Source: CAD feature listing. Evaluate the final solid. Frame: model axes, mm. Face numbers are marked on the shaded views. A direction names the side the tool comes from. Coordinates: 2 decimals unless noted, no trailing zeros. Loops run counter-clockwise (first coordinate to the right, second up) from the corner with the lowest first, then second, coordinate; pieces in that order, holes last. Notation, with made-up numbers: M 78,7.5 L 129,7.5 A19 ccw 129,35.5 Z; hole C 54.25,-7.75 d10. An arc over 180 degrees is marked long. Write each question's results on one line, items separated by ' | '. Start each with the question number.
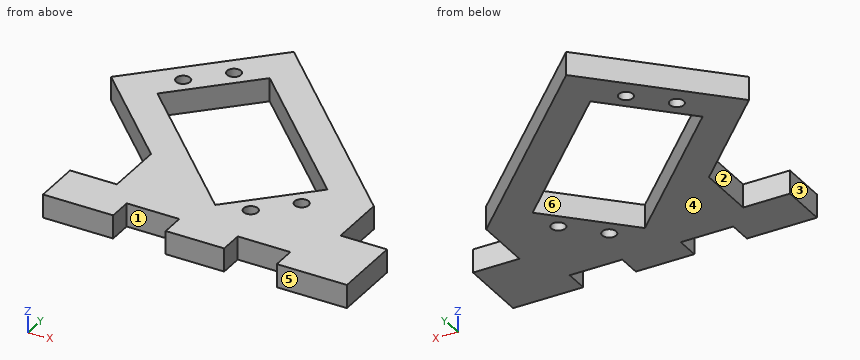
from build123d import *

# Parameters (mm, degrees)
SKETCH_1_R      = 1.5
EXTRUDE_1_DEPTH = 5


with BuildPart() as part:
    # 草图1 → 凸台-拉伸1 (new body)
    with BuildSketch(Plane.XY):
        Polygon((-12.648598414, -34.707783696), (-27.648598414, -34.707783696), (-27.648598414, -24.707783696), (-17.648598414, -24.707783696), (-17.648598414, -12.085840997), (-37.977918373, 8.243478962), (-13.229181032, 32.992216304), (27.420818968, -7.657783696), (27.420818968, -19.907783696), (37.351401586, -19.907783696), (37.351401586, -34.707783696), (22.351401586, -34.707783696), (22.351401586, -29.707783696), (11.101401586, -29.707783696), (11.101401586, -34.707783696), (-1.398598414, -34.707783696), (-1.398598414, -29.707783696), (-12.648598414, -29.707783696), align=None)
        with Locations((-19.009778968, 20.918368015)):
            Circle(SKETCH_1_R, mode=Mode.SUBTRACT)
        with Locations((-25.904070084, 14.024076898)):
            Circle(SKETCH_1_R, mode=Mode.SUBTRACT)
        with Locations((15.355610598, -13.447021551)):
            Circle(SKETCH_1_R, mode=Mode.SUBTRACT)
        with Locations((8.461319481, -20.341312667)):
            Circle(SKETCH_1_R, mode=Mode.SUBTRACT)
        Polygon((-27.548093351, 7.359595486), (1.796838069, -21.985335933), (16.999633864, -6.782540138), (-12.345297555, 22.562391281), align=None, mode=Mode.SUBTRACT)
    extrude(amount=EXTRUDE_1_DEPTH)


solid = part.part
Item 1: Line query: probe 1 along X at (y, z) = (-13.5, 3.6); probe 2 along Y at (x, z) = (-19.5, 0.85); probe 3 along X at (y, z) = (-28, 2). Output: solid intervals per line, ascending.
Item 2: Access query for the marked faces 1, 2 and 3. Directions: +Z, -Z, +X, -X, +Y, -Y. A direction counts if a zero-diameter tool reaches every point of the face in a straight line with its end or side. Return the directions, or none.
Item 3: First-contact query: pin 1 Ø2 at (x, z) = (18, 1.5) entering from +Y; pin 2 Ø2.5 at (y, z) = (-31.5, 1.5) entering from -X; pin 3 Ø3 at (y, z) = (25, 3) entering from -X. Flat tips, straight axial feed; report the tip coordinate or a pass-through.
Item 4: Cut plane C-C (z = 2.05). Output: boundary loops of the cut face in (x, y).
Item 5: Cut plane A-A (x = -10). Output: boundary loops of the cut face in (y, z).
Item 6: Cut plane B-B (y = 10.5). Output: boundary loops of the cut face in (x, z), then the cut area to 3 significant figures.
Item 7: Cut plane D-D (x = -19.5). Output: boundary loops of the cut face in (y, z), then the cut area to 3 significant figures.
Item 8: Mould query, pull axis Y, two halves, no side actions, for the marked faces 4, 5 and 6. Classes: +Y half, -Y half, draft (parallel to the pull), parting line (faces both ways), or undercut.
Response values:
1) probe 1: x = -17.65 to -6.69, 10.28 to 13.86, 16.85 to 27.42 | probe 2: y = -34.71 to -24.71, -10.23 to -0.69, 15.41 to 19.5, 22.34 to 26.72 | probe 3: x = -27.65 to 37.35
2) face 1: +Z, -Z, -Y | face 2: +Z, -Z, -X | face 3: +Z, -Z, -X, -Y
3) pin 1: stops at y = 2.76 | pin 2: stops at x = -27.65 | pin 3: stops at x = -22.72
4) outline: M -37.98,8.24 L -17.65,-12.09 L -17.65,-24.71 L -27.65,-24.71 L -27.65,-34.71 L -12.65,-34.71 L -12.65,-29.71 L -1.4,-29.71 L -1.4,-34.71 L 11.1,-34.71 L 11.1,-29.71 L 22.35,-29.71 L 22.35,-34.71 L 37.35,-34.71 L 37.35,-19.91 L 27.42,-19.91 L 27.42,-7.66 L -13.23,32.99 Z; hole M -27.55,7.36 L 1.8,-21.99 L 17,-6.78 L -12.35,22.56 Z; hole C -25.9,14.02 d3; hole C -19.01,20.92 d3; hole C 8.46,-20.34 d3; hole C 15.36,-13.45 d3
5) outline: M -29.71,0 L -10.19,0 L -10.19,5 L -29.71,5 Z; M 20.22,0 L 29.76,0 L 29.76,5 L 20.22,5 Z
6) outline: M -35.72,0 L -24.41,0 L -24.41,5 L -35.72,5 Z; M -0.28,0 L 9.26,0 L 9.26,5 L -0.28,5 Z | area: 104 mm2
7) outline: M -34.71,0 L -24.71,0 L -24.71,5 L -34.71,5 Z; M -10.23,0 L -0.69,0 L -0.69,5 L -10.23,5 Z; M 15.41,0 L 19.5,0 L 19.5,5 L 15.41,5 Z; M 22.34,0 L 26.72,0 L 26.72,5 L 22.34,5 Z | area: 140 mm2
8) face 4: draft | face 5: -Y half | face 6: undercut
